from build123d import *

# Parameters (mm, degrees)
SKETCH_1_W                = 36
SKETCH_1_H                = 39
EXTRUDE_1_DEPTH           = 10
SKETCH_2_W                = 32
SKETCH_2_H                = 39
CUT_EXTRUDE_1_DEPTH       = 1.5
SKETCH_3_W                = 12
SKETCH_3_H                = 28
EXTRUDE_2_DEPTH           = 65
HOLE_WIZARD_5_0_5_1_D     = 5
HOLE_WIZARD_5_0_5_1_DEPTH = 10


with BuildPart() as part:
    # 草图1 → 凸台-拉伸1 (new body)
    with BuildSketch(Plane.XY):
        Rectangle(SKETCH_1_W, SKETCH_1_H)
    extrude(amount=EXTRUDE_1_DEPTH)

    # 草图2 → 切除-拉伸1 (cut)
    with BuildSketch(Plane.XY.offset(10)):
        Rectangle(SKETCH_2_W, SKETCH_2_H)
    extrude(amount=-CUT_EXTRUDE_1_DEPTH, mode=Mode.SUBTRACT)

    # 草图3 → 凸台-拉伸2 (add)
    with BuildSketch(Plane(origin=(0, 0, 0), x_dir=(-1, 0, 0), z_dir=(0, 0, -1))):
        with Locations((0, -5.5)):
            Rectangle(SKETCH_3_W, SKETCH_3_H)
    extrude(amount=EXTRUDE_2_DEPTH)

    # Ø5.0 (5) 直径孔1
    with Locations(Plane(origin=(0, 0, 0), x_dir=(-1, 0, 0), z_dir=(0, 0, -1))):
        with Locations((-12, 9.7), (12, 9.7), (12, -10.3), (-12, -10.3)):
            Hole(HOLE_WIZARD_5_0_5_1_D / 2, depth=HOLE_WIZARD_5_0_5_1_DEPTH)


solid = part.part
Check sheet for the modelled part. Datum: model origin and axes. Units: mm. A direction names the side the tool comes from. Round coordinates to 2 decimals unless told otherwise and drop trailing zeros. Order: outer loops, then holes, each group sorted by start corner. A loop starts at its lowest first (then second) coordinate and runs counter-clockwise, first axis right, second up.
Q1. Draft check along Y on faces 5 (the face through (-13.84, 11.39, 4.31)), 6 (the face through (9.5, -10.2, 4.3)), 7 (the face through (0, -5, -65)), 8 (the face through (0, 19.5, 5)). Enter one of: pulls with the +Y half, pulls with the -Y half, needs draft (parallel to the pull), parting line crosses it, or undercut.
Filled sheet:
face 5: undercut
face 6: undercut
face 7: needs draft
face 8: pulls with the +Y half
Q2. Set-up check for faces 1 (the face through (6, -6, -32)), 2 (the face through (-6, -6, -32)), 3 (the face through (16, 0, 9)), 4 (the face through (0, 8.5, -32)): record each of +Z, -Z, +X, -X, +Y, -Y from which the full face is reachable in a straight line by a thin tool's end or side.
Filled sheet:
face 1: -Z, +X, +Y, -Y
face 2: -Z, -X, +Y, -Y
face 3: +Z, +Y, -Y
face 4: -Z, +X, -X, +Y
Q3. Scan lines: L1, parallel to Y at x = -12, z = 4; L2, parallel to X at y = 9, z = 2; L3, parallel to Z at x = 1.5, y = -8.5. Record each from-to range of solid material in increasing order.
Filled sheet:
L1: y = -19.5 to -12.8, -7.8 to 7.2, 12.2 to 19.5
L2: x = -18 to -14.4, -9.6 to 9.6, 14.4 to 18
L3: z = -65 to 8.5
Q4. Cross-section at C-C, the plane x = -5. Enter the section's corners in (y, z).
Filled sheet:
outline: (-19.5, -65) - (8.5, -65) - (8.5, 0) - (19.5, 0) - (19.5, 8.5) - (-19.5, 8.5) - close
Q5. Depth check by flat-ended pin: P1, Ø12, axis at x = -10.5, z = -2.5, coming from the +Y side; P2, Ø6, axis at x = -10, y = 12.5, coming from the +Z side; P3, Ø22.5, axis at y = -1, z = -23, coming from the -X side; P4, Ø2, axis at y = -15.5, z = -13.5, coming from the +X side. Enter the tip coordinate at first touch or a pass-through.
Filled sheet:
P1: stops at y = 19.5
P2: stops at z = 8.5
P3: stops at x = -6
P4: stops at x = 6
Q6. Cross-section at D-D, the plane z = -44. Enter the section's corners in (x, y), plus the area to 3 significant figures.
Filled sheet:
outline: (-6, -19.5) - (6, -19.5) - (6, 8.5) - (-6, 8.5) - close
area: 336 mm2
Q7. Cross-section at A-A, the plane x = -12. Enter the section's corners in (y, z), plus the area to 4 significant figures.
Filled sheet:
outline: (-19.5, 0) - (-12.8, 0) - (-12.8, 8.5) - (-19.5, 8.5) - close; (-7.8, 0) - (7.2, 0) - (7.2, 8.5) - (-7.8, 8.5) - close; (12.2, 0) - (19.5, 0) - (19.5, 8.5) - (12.2, 8.5) - close
area: 246.5 mm2
Q8. Cross-section at B-B, the plane y = 0. Enter the section's corners in (x, z).
Filled sheet:
outline: (-18, 0) - (-6, 0) - (-6, -65) - (6, -65) - (6, 0) - (18, 0) - (18, 10) - (16, 10) - (16, 8.5) - (-16, 8.5) - (-16, 10) - (-18, 10) - close
